from build123d import *

# Parameters (mm, degrees)
SKETCH_1_R          = 7.5
EXTRUDE_1_DEPTH     = 100
EXTRUDE_START       = -25.5
SKETCH_2_R          = 9
EXTRUDE_2_DEPTH     = 3
EXTRUDE_START_2     = -28.5
SKETCH_3_R          = 9
EXTRUDE_3_DEPTH     = 3
EXTRUDE_START_3     = 40
SKETCH_4_R          = 7.5
EXTRUDE_4_DEPTH     = 40
SKETCH_5_R          = 10
CUT_EXTRUDE_2_DEPTH = 81.5


with BuildPart() as part:
    # 草图1 → 凸台-拉伸1 (new body)
    with BuildSketch(Plane.XY):
        Circle(SKETCH_1_R)
    extrude(amount=EXTRUDE_1_DEPTH)

    # 草图2 → 凸台-拉伸2 (add)
    with BuildSketch(Plane.XY.offset(100).offset(EXTRUDE_START)):
        Circle(SKETCH_2_R)
    extrude(amount=-EXTRUDE_2_DEPTH)

    # 草图3 → 凸台-拉伸3 (add)
    with BuildSketch(Plane(origin=(0, 0, 0), x_dir=(-1, 0, 0), z_dir=(0, 0, -1)).offset(EXTRUDE_START_2)):
        with Locations(Location((0, 0, 0), (0, 0, 180))):
            Circle(SKETCH_3_R)
    extrude(amount=EXTRUDE_3_DEPTH)

    # 草图4 → 凸台-拉伸4 (add)
    with BuildSketch(Plane(origin=(0, 0, 0), x_dir=(-1, 0, 0), z_dir=(0, 0, -1)).offset(EXTRUDE_START_3)):
        Circle(SKETCH_4_R)
    extrude(amount=-EXTRUDE_4_DEPTH)

    # 草图5 → 切除-拉伸2 (cut)
    with BuildSketch(Plane(origin=(0, 0, -40), x_dir=(-1, 0, 0), z_dir=(0, 0, -1))):
        Circle(SKETCH_5_R)
    extrude(amount=-CUT_EXTRUDE_2_DEPTH, mode=Mode.SUBTRACT)


solid = part.part
Check sheet for the modelled part. Datum: model origin and axes. Units: mm. A direction names the side the tool comes from. Coordinates: 2 decimals unless noted, no trailing zeros. Loops run counter-clockwise (first coordinate to the right, second up) from the corner with the lowest first, then second, coordinate; pieces in that order, holes last. Notation, with made-up numbers: (37, -15.75) -> (65, -15.75) arc R33 cw to (65, 19.25) -> close; hole circle Ø2 at (-3, 22). An arc over 180 degrees is marked (long way). Write item = value, one per line. Start each with the question number.
1. Section check C-C on z = 56.5. Record the cut outline in (x, y), then the cut area to 3 significant figures.
2. Material ranges on line 1 (Z direction, x = -4.75, y = 7.25); line 2 (Y direction, x = -2.75, z = 73.5); line 3 (Y direction, x = 2, z = 59.5), recorded low to high.
3. Section check A-A on x = 0. Record the cut outline in (y, z).
4. Depth check by flat-ended pin: P1, Ø2, axis at y = 4.5, z = 78, coming from the +X side; P2, Ø3, axis at x = -6, z = 56, coming from the +Y side; P3, Ø2, axis at y = 1, z = 67, coming from the +X side. Enter the tip coordinate at first touch or a pass-through.
5. Tool access check on faces 1 (the cylindrical face through (-7.493, 0.33, 56.29)), 2 (the cylindrical face through (-1.172, 8.923, 73.021)), 3 (the flat face through (-2, 7.4, 74.5)). Record the directions out of +Z, -Z, +X, -X, +Y, -Y that give a thin tool (end or side, any length) a straight path to the whole face; none if there is none.
Responses:
q1.outline = circle Ø15 at (0, 0)
q1.area = 177 mm2
q2.line_1 = 71.5 to 74.5
q2.line_2 = -8.57 to 8.57
q2.line_3 = -7.23 to 7.23
q3.outline = (-9, 71.5) -> (-7.5, 71.5) -> (-7.5, 41.5) -> (7.5, 41.5) -> (7.5, 71.5) -> (9, 71.5) -> (9, 74.5) -> (7.5, 74.5) -> (7.5, 100) -> (-7.5, 100) -> (-7.5, 74.5) -> (-9, 74.5) -> close
q4.P1 = 6.63
q4.P2 = 6
q4.P3 = 7.5
q5.face_1 = -Z
q5.face_2 = +Z, -Z
q5.face_3 = +Z
